from build123d import *

# Parameters (mm, degrees)
SKETCH2_R           = 20
SKETCH2_R_2         = 3.5
BOSS_EXTRUDE1_DEPTH = 2
FILLET1_R           = 5
FILLET2_R           = 5


with BuildPart() as part:
    # Sketch2 → Boss-Extrude1 (new body)
    with BuildSketch(Plane(origin=(0, 0, 0), x_dir=(1, 0, 0), z_dir=(0, 1, 0))):
        with BuildLine():
            ThreePointArc((-27.733348113, 16.944361965), (-32.5, 0), (-27.733348113, -16.944361965))
            ThreePointArc((-27.733348113, -16.944361965), (-29.69848481, -29.69848481), (-16.944361965, -27.733348113))
            ThreePointArc((-16.944361965, -27.733348113), (0, -32.5), (16.944361965, -27.733348113))
            ThreePointArc((16.944361965, -27.733348113), (29.69848481, -29.69848481), (27.733348113, -16.944361965))
            ThreePointArc((27.733348113, -16.944361965), (32.5, 0), (27.733348113, 16.944361965))
            ThreePointArc((27.733348113, 16.944361965), (29.69848481, 29.69848481), (16.944361965, 27.733348113))
            ThreePointArc((16.944361965, 27.733348113), (0, 32.5), (-16.944361965, 27.733348113))
            ThreePointArc((-16.944361965, 27.733348113), (-29.69848481, 29.69848481), (-27.733348113, 16.944361965))
        make_face()
        with Locations(Location((0, 0, 0), (0, 0, 270))):
            Circle(SKETCH2_R, mode=Mode.SUBTRACT)
        with Locations(Location((-24.04163056, 24.04163056, 0), (0, 0, 270))):
            Circle(SKETCH2_R_2, mode=Mode.SUBTRACT)
        with Locations(Location((24.04163056, 24.04163056, 0), (0, 0, 270))):
            Circle(SKETCH2_R_2, mode=Mode.SUBTRACT)
        with Locations(Location((24.04163056, -24.04163056, 0), (0, 0, 270))):
            Circle(SKETCH2_R_2, mode=Mode.SUBTRACT)
        with Locations(Location((-24.04163056, -24.04163056, 0), (0, 0, 270))):
            Circle(SKETCH2_R_2, mode=Mode.SUBTRACT)
    extrude(amount=BOSS_EXTRUDE1_DEPTH)

    # Fillet1
    fillet1_edges = [part.edges().sort_by_distance(p)[0] for p in [
        (16.944361965, 1, -27.733348113),
        (27.733348113, 1, -16.944361965),
        (27.733348113, 1, 16.944361965),
        (16.944361965, 1, 27.733348113),
        (-16.944361965, 1, 27.733348113),
        (-27.733348113, 1, 16.944361965),
        (-27.733348113, 1, -16.944361965),
    ]]
    fillet(fillet1_edges, radius=FILLET1_R)

    # Fillet2
    fillet2_edges = [part.edges().sort_by_distance(p)[0] for p in [
        (-16.944361965, 1, -27.733348113),
    ]]
    fillet(fillet2_edges, radius=FILLET2_R)


solid = part.part
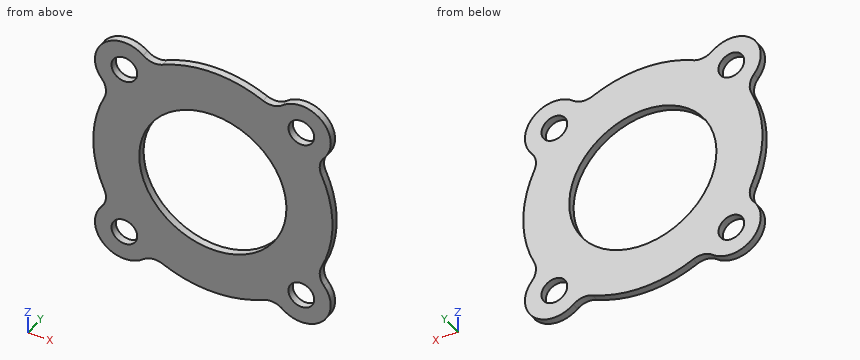
CAD build for the part. Positions are in the model's coordinates, mm. Round coordinates to 2 decimals unless told otherwise and drop trailing zeros. Write each loop counter-clockwise with the first axis right and the second up, starting at its lowest first coordinate (ties: lowest second). Pieces come first, ordered by that corner, then holes.
(1) Slice it at B-B, the plane x = 0. Write the cut outline in (y, z).
(2) Slice it at D-D, the plane x = 22. Write the cut outline in (y, z).
(3) Probe line 1 along X through (y, z) = (0.7, -0.5); line 2 along X through (y, z) = (0.7, 26); line 3 along Z through (x, y) = (14, 1.4). List the from-to ranges inside material, lowest first.
(4) Slice it at A-A, the plane z = 0. Write the cut outline in (x, y), and give its area (3 significant figures).
(5) Drop flat-ended pins along their axis: P1, Ø6.5, axis at x = 24.04, z = 24.04, coming from the -Y side; P2, Ø1, axis at x = 24, y = 1, coming from the -Z side; P3, Ø1, axis at y = 1, z = 18, coming from the -X side. Give the stop position or say it passes through.
(6) Slice it at C-C, the plane z = 23.5. Write the cut outline in (x, y), and give its area (3 significant figures).
From the geometry:
1. outline: (0, -32.5) - (2, -32.5) - (2, -20) - (0, -20) - close; (0, 20) - (2, 20) - (2, 32.5) - (0, 32.5) - close
2. outline: (0, -31.78) - (2, -31.78) - (2, -26.88) - (0, -26.88) - close; (0, -21.2) - (2, -21.2) - (2, 21.2) - (0, 21.2) - close; (0, 26.88) - (2, 26.88) - (2, 31.78) - (0, 31.78) - close
3. line 1: x = -32.5 to -19.99, 19.99 to 32.5
3. line 2: x = -31.8 to -26.94, -21.14 to 21.14, 26.94 to 31.8
3. line 3: z = -29.35 to -14.28, 14.28 to 29.35
4. outline: (-32.5, 0) - (-20, 0) - (-20, 2) - (-32.5, 2) - close; (20, 0) - (32.5, 0) - (32.5, 2) - (20, 2) - close
4. area: 50.0 mm2
5. P1: passes through
5. P2: stops at z = -32.04
5. P3: stops at x = -29.88
6. outline: (-32.02, 0) - (-27.5, 0) - (-27.5, 2) - (-32.02, 2) - close; (-20.58, 0) - (20.58, 0) - (20.58, 2) - (-20.58, 2) - close; (27.5, 0) - (32.02, 0) - (32.02, 2) - (27.5, 2) - close
6. area: 100 mm2
